Design review of the part built by this model. Coordinates are the model's own, in mm. Coordinates: 2 decimals unless noted, no trailing zeros. Loops run counter-clockwise (first coordinate to the right, second up) from the corner with the lowest first, then second, coordinate; pieces in that order, holes last. Notation, with made-up numbers: M -38.75,55 L 6.25,55 A22 ccw 6.25,64 Z; hole C 20,7.25 d11. An arc over 180 degrees is marked long. Answer as a JSON object with one key per item and string values. Group by question number.
1. Insertion check: pin 1 (1 mm diameter, centred on y = 0, z = 695, fed in from +X); pin 2 (1.5 mm diameter, centred on y = -0.5, z = 153.5, fed in from -X). Each pin has a flat end and moves straight along its axis. Give the tip position at first contact, or say it passes through.
2. Consider section B-B (x = -214.5). State the section outline as (y, z) points.
3. Consider section A-A (y = 0). State the section outline as (x, z) points.
4. To check wall thickness, follow probe 1 along X at (y, z) = (0.75, 360); probe 2 along Z at (x, y) = (-20.5, 0); probe 3 along Z at (x, y) = (-210.5, 1.5). State the ranges of each line that lie inside material, in increasing order.
5. Consider section C-C (z = 428.5). State the section outline as (x, y) points, then the cut area to 3 significant figures.
from build123d import *

# Parameters (mm, degrees)
SKETCH2_R = 3


with BuildPart() as part:
    # Sweep1: sweep along a path in Sketch1
    with BuildLine(Plane(origin=(0, 0, 0), x_dir=(1, 0, 0), z_dir=(0, 1, 0))) as sweep1_path:
        Line((0, 0), (-432.5, 0))
        ThreePointArc((-432.5, 0), (-438.863961031, -2.636038969), (-441.5, -9))
        Line((-441.5, -9), (-441.5, -705.408118144))
        ThreePointArc((-441.5, -705.408118144), (-440.858887638, -708.744133349), (-439.026889456, -711.604868424))
        Line((-439.026889456, -711.604868424), (-280.861457438, -878.19675028))
        ThreePointArc((-280.861457438, -878.19675028), (-277.886275141, -880.269545106), (-274.334567982, -881))
        Line((-274.334567982, -881), (0, -881))
    # Sketch2 → Sweep1 (sweep)
    with BuildSketch(Plane(origin=(0, 0, 0), x_dir=(0, 0, -1), z_dir=(1, 0, 0))):
        Circle(SKETCH2_R)
    sweep(path=sweep1_path.line)


solid = part.part
Findings below:
{
 "1": {"pin 1": "stops at x = -438.5", "pin 2": "stops at x = -444.5"},
 "2": {"outline": "C 0,0 d6; C 0,881 d6"},
 "3": {"outline": "M -444.5,9 A12 ccw -432.5,-3 L 0,-3 L 0,3 L -432.5,3 A6 cw -438.5,9 L -438.5,705.41 A6 cw -436.85,709.54 L -278.69,876.13 A6 cw -274.33,878 L 0,878 L 0,884 L -274.33,884 A12 ccw -283.04,880.26 L -441.2,713.67 A12 ccw -444.5,705.41 Z"},
 "4": {"probe 1": "x = -444.4 to -438.6", "probe 2": "z = -3 to 3, 878 to 884", "probe 3": "z = -2.6 to 2.6, 878.4 to 883.6"},
 "5": {"outline": "C -441.5,0 d6", "area": "28.3 mm^2"}
}
